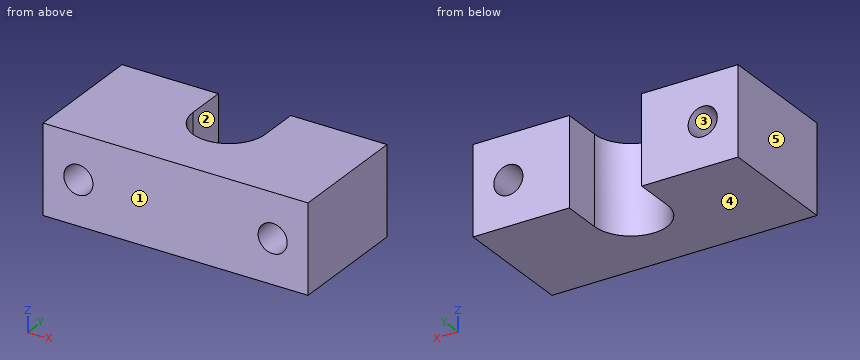
```python
from build123d import *

# Parameters (mm, degrees)
SKETCH1_W           = 30
SKETCH1_H           = 14
BOSS_EXTRUDE1_DEPTH = 5
CUT_EXTRUDE1_DEPTH  = 20.339079606
M4_TAPPED_HOLE1_D   = 3.3


with BuildPart() as part:
    # Sketch1 → Boss-Extrude1 (new, symmetric)
    with BuildSketch(Plane.XY):
        Rectangle(SKETCH1_W, SKETCH1_H)
    extrude(amount=BOSS_EXTRUDE1_DEPTH, both=True)

    # Sketch2 → Cut-Extrude1 (cut, through all)
    with BuildSketch(Plane.XY.offset(5)):
        with BuildLine():
            Line((4.1, 7), (4.1, 2.5))
            ThreePointArc((4.1, 2.5), (0, -1.6), (-4.1, 2.5))
            Line((-4.1, 2.5), (-4.1, 7))
            ThreePointArc((-4.1, 7), (0, 11.1), (4.1, 7))
        make_face()
    extrude(amount=-CUT_EXTRUDE1_DEPTH, mode=Mode.SUBTRACT)

    # M4 Tapped Hole1 (through all)
    with Locations(Plane(origin=(0, 7, 0), x_dir=(1, 0, 0), z_dir=(0, 1, 0))):
        with Locations((-11, 0), (11, 0)):
            Hole(M4_TAPPED_HOLE1_D / 2)


solid = part.part
```
Model file for the job. Use its own axes, mm. Face numbers are marked on the shaded views. A direction names the side the tool comes from. Round coordinates to 2 decimals unless told otherwise and drop trailing zeros. Loops run counter-clockwise (first coordinate to the right, second up) from the corner with the lowest first, then second, coordinate; pieces in that order, holes last. Notation, with made-up numbers: M 30,-6 L 38,-6 A14 cw 38,5 Z; hole C 19,25 d3. An arc over 180 degrees is marked long. Put each result on its own line as item: value. Start each with the question number.
Item 1: Drill centre lines: line 1 along X through (y, z) = (4.25, -3); line 2 along Z through (x, y) = (-11, -4); line 3 along X through (y, z) = (-0.5, -1.25). Where is each one in solid material? Low to high.
Item 2: 3-axis set-ups, long thin cutter, end or side, ignore diameter. For the marked faces 1 and 2: which of +Z, -Z, +X, -X, +Y, -Y reach the whole face in a straight line?
Item 3: Cut at B-B (z = 0). List the corners of the cut face in (x, y), then the cut area to 3 significant figures.
Item 4: Mould opens along Z. For the marked faces 3, 4 and 5 say: released by +Z, released by -Z, zero draft, split by the parting line, or undercut.
Item 5: Cut at C-C (x = 11). List the corners of the cut face in (y, z), then the cut area to 3 significant figures.
Item 6: Cut at D-D (y = -2.5). List the corners of the cut face in (x, z).
Item 7: Drop a flat-ended pin along its axis: P1, Ø2.5, axis at x = 11, z = 0, coming from the -Y side. Give the stop position or say it passes through.
Item 8: Cut at A-A (y = 6.25). List the corners of the cut face in (x, z), then the cut area to 3 significant figures.
Answer block:
1. line 1: -15 to -4.1, 4.1 to 15
1. line 2: -5 to -1.65, 1.65 to 5
1. line 3: -15 to -12.08, -9.92 to -2.79, 2.79 to 9.92, 12.08 to 15
2. face 1: +Z, -Z, +X, -X, -Y
2. face 2: +Z, -Z, +Y
3. outline: M -15,-7 L -12.65,-7 L -12.65,7 L -15,7 Z; M -9.35,-7 L 9.35,-7 L 9.35,7 L 4.1,7 L 4.1,2.5 A4.1 cw -4.1,2.5 L -4.1,7 L -9.35,7 Z; M 12.65,-7 L 15,-7 L 15,7 L 12.65,7 Z
3. area: 264 mm2
4. face 3: undercut
4. face 4: released by -Z
4. face 5: zero draft
5. outline: M -7,-5 L 7,-5 L 7,-1.65 L -7,-1.65 Z; M -7,1.65 L 7,1.65 L 7,5 L -7,5 Z
5. area: 93.8 mm2
6. outline: M -15,-5 L 15,-5 L 15,5 L -15,5 Z; hole C -11,0 d3.3; hole C 11,0 d3.3
7. P1: through
8. outline: M -15,-5 L -4.1,-5 L -4.1,5 L -15,5 Z; M 4.1,-5 L 15,-5 L 15,5 L 4.1,5 Z; hole C -11,0 d3.3; hole C 11,0 d3.3
8. area: 201 mm2
